Here's how the part is built. I have some questions about the finished solid (model axes, mm). Round coordinates to 2 decimals unless told otherwise and drop trailing zeros. Write each loop counter-clockwise with the first axis right and the second up, starting at its lowest first coordinate (ties: lowest second). Pieces come first, ordered by that corner, then holes. Notation, with made-up numbers: (14, 87.5) - (44, 87.5) arc R25 cw to (44, 122.5) - close; hole circle Ø1 at (52.25, 88). An arc over 180 degrees is marked (long way). One line per item, written item: value. Start each with the question number.
Item 1: Imagine slicing it at A-A, the plane y = 415.5. Please give me the cut outline in (x, z), then the cut area to 3 significant figures.
Item 2: If I drill on line 1 (Y direction, x = -1, z = 0); line 2 (Y direction, x = 2.5, z = 0.5); line 3 (Y direction, x = 4.5, z = 5.5), over which ranges is the centre line in solid material (lowest first)?
Item 3: For P1, Ø1, axis at y = 412.5, z = 3, coming from the +X side; P2, Ø8, axis at x = -0.5, y = 176, coming from the -Z side; P3, Ø2, axis at y = 373, z = -1.5, coming from the +X side; P4, Ø2, axis at x = -5, y = 284, coming from the -Z side, each with a flat end and sliding along its axis, tell me the tip position at first contact or that it passes through.
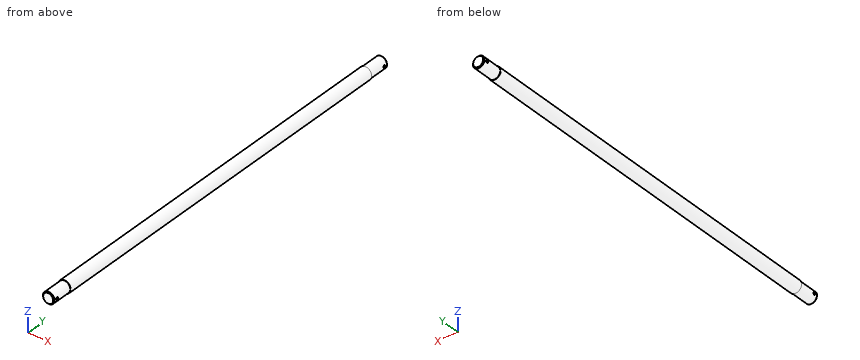
```python
from build123d import *

# Parameters (mm, degrees)
CHAMFER1_SIZE           = 1
CUT_EXTRUDE1_DEPTH      = 511.110282194
CUT_EXTRUDE1_DEPTH_BACK = 511.110282194
SKETCH3_R               = 1.5


with BuildPart() as part:
    # Sketch1 → Revolve1 (revolve)
    with BuildSketch(Plane.XY, mode=Mode.PRIVATE) as revolve1_sk:
        Polygon((0, 0), (7, 0), (7, 25), (7.5, 25), (7.5, 485), (7, 485), (7, 510), (0, 510), align=None)
    revolve(revolve1_sk.sketch.rotate(Axis((0, 0, 0), (0, -1, 0)), 90), axis=Axis((0, 0, 0), (0, -1, 0)))

    # Chamfer1
    chamfer1_edges = [part.edges().sort_by_distance(p)[0] for p in [
        (0, 510, -7),
        (0, 0, -7),
    ]]
    chamfer(chamfer1_edges, length=CHAMFER1_SIZE)

    # Sketch3 → Cut-Extrude1 (cut, two sides: drawn at the far end of the back side and taken through both)
    with BuildSketch(Plane(origin=(0, 0, 0), x_dir=(0, 0, -1), z_dir=(1, 0, 0)).offset(-CUT_EXTRUDE1_DEPTH_BACK)):
        with Locations((0, 505)):
            Circle(SKETCH3_R)
        with Locations((0, 5)):
            Circle(SKETCH3_R)
    extrude(amount=CUT_EXTRUDE1_DEPTH + CUT_EXTRUDE1_DEPTH_BACK, mode=Mode.SUBTRACT)


solid = part.part
```
Values follow:
1. outline: circle Ø15 at (0, 0)
1. area: 177 mm^2
2. line 1: y = 0 to 3.5, 6.5 to 503.5, 506.5 to 510
2. line 2: y = 0 to 3.59, 6.41 to 503.59, 506.41 to 510
2. line 3: y = 25 to 485
3. P1: stops at x = 7.07
3. P2: stops at z = -7.5
3. P3: stops at x = 7.48
3. P4: stops at z = -6.34
